Read the model definition and answer for the solid it produces. Units are mm, in the model's axes. Face numbers are marked on the shaded views. Give positions to 0.01 mm unless a question says otherwise; leave off trailing zeros. Loops run counter-clockwise (first coordinate to the right, second up) from the corner with the lowest first, then second, coordinate; pieces in that order, holes last. Notation, with made-up numbers: (66, 46) -> (105, 46) arc R13 cw to (105, 52) -> close; hole circle Ø10 at (-27.75, 63.5). An arc over 180 degrees is marked (long way). Write each question's results on one line, items separated by ' | '. Start each with the question number.
Item 1: Each of these flat-tipped pins is pushed along its axis until it touches: P1, Ø9, axis at x = 21, y = 34.3, coming from the +Z side; P2, Ø2.5, axis at x = 73.5, y = 6, coming from the +Z side. Where does it stop, or does it pass through?
Item 2: Section C-C on z = -6.5 is taken. State how many separate pieces and enclosed holes the cut face has, and give its area (3 significant figures).
Item 3: Section B-B on y = 21.8 is taken. Write down the section's boundary in (x, z), and give its area (3 significant figures).
Item 4: Section A-A on x = 21 is taken. Write down the section's boundary in (y, z).
Item 5: Find the intervals of material crossed by line 1 (Y direction, x = 75, z = -2.1); line 2 (Y direction, x = 36.5, z = -3); line 3 (X direction, y = 9, z = -2), in increasing order.
Item 6: Determine the mould class of the marked faces 1, 2 and 3 for opening direction X: +X half, -X half, draft (parallel to the pull), parting line (faces both ways), or undercut.
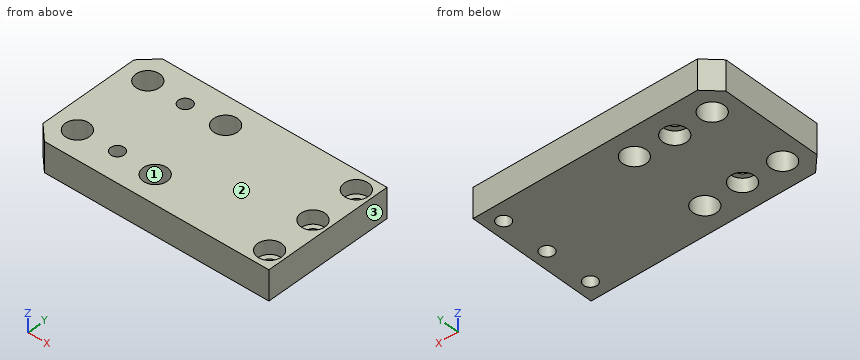
```python
from build123d import *

# Parameters (mm, degrees)
SKETCH_1_W                   = 80
SKETCH_1_H                   = 10
EXTRUDE_1_DEPTH              = 43.6
CHAMFER_1_SIZE               = 5
HOLE_WIZARD_8_0_8_1_D        = 8
HOLE_WIZARD_M4_1_D           = 4.5
HOLE_WIZARD_M4_1_CBORE_D     = 8
HOLE_WIZARD_M4_1_CBORE_DEPTH = 4.6
HOLE_WIZARD_M4_2_D           = 4.5
HOLE_WIZARD_M4_2_CBORE_D     = 8
HOLE_WIZARD_M4_2_CBORE_DEPTH = 4.6


with BuildPart() as part:
    # 草图1 → 凸台-拉伸1 (new body)
    with BuildSketch(Plane(origin=(0, 0, 0), x_dir=(1, 0, 0), z_dir=(0, 1, 0))):
        with Locations((40, 5)):
            Rectangle(SKETCH_1_W, SKETCH_1_H)
    extrude(amount=EXTRUDE_1_DEPTH)

    # 倒角1
    chamfer_1_edges = [part.edges().sort_by_distance(p)[0] for p in [
        (0, 43.6, -5),
        (0, 0, -5),
    ]]
    chamfer(chamfer_1_edges, length=CHAMFER_1_SIZE)

    # Ø8.0 (8) 直径孔1 (through all)
    with Locations(Plane(origin=(0, 0, -10), x_dir=(-1, 0, 0), z_dir=(0, 0, -1))):
        with Locations((-34.042753413, 34.8), (-8.042753413, 34.8), (-8.042753413, 8.8), (-34.042753413, 8.8)):
            Hole(HOLE_WIZARD_8_0_8_1_D / 2)

    # M4 六角圆柱头螺钉的柱形沉头孔1 (through all)
    with Locations(Plane(origin=(0, 0, -10), x_dir=(-1, 0, 0), z_dir=(0, 0, -1))):
        with Locations((-21, 34.3), (-21, 9.3)):
            CounterBoreHole(HOLE_WIZARD_M4_1_D / 2, HOLE_WIZARD_M4_1_CBORE_D / 2, HOLE_WIZARD_M4_1_CBORE_DEPTH)

    # M4 六角圆柱头螺钉的柱形沉头孔2 (through all)
    with Locations(Plane.XY):
        with Locations((75, 37.8), (75, 5.8), (75, 21.8)):
            CounterBoreHole(HOLE_WIZARD_M4_2_D / 2, HOLE_WIZARD_M4_2_CBORE_D / 2, HOLE_WIZARD_M4_2_CBORE_DEPTH)


solid = part.part
```
Findings:
1) P1: z = 0 | P2: z = -4.6
2) separate pieces: 1 | enclosed holes: 9 | area: 3,110 mm2
3) outline: (0, -10) -> (72.75, -10) -> (72.75, -4.6) -> (71, -4.6) -> (71, 0) -> (0, 0) -> close; (77.25, -10) -> (80, -10) -> (80, 0) -> (79, 0) -> (79, -4.6) -> (77.25, -4.6) -> close | area: 739 mm2
4) outline: (0, -10) -> (5.3, -10) -> (5.3, -5.4) -> (7.05, -5.4) -> (7.05, 0) -> (0, 0) -> close; (11.55, -5.4) -> (13.3, -5.4) -> (13.3, -10) -> (30.3, -10) -> (30.3, -5.4) -> (32.05, -5.4) -> (32.05, 0) -> (11.55, 0) -> close; (36.55, -5.4) -> (38.3, -5.4) -> (38.3, -10) -> (43.6, -10) -> (43.6, 0) -> (36.55, 0) -> close
5) line 1: 0 to 1.8, 9.8 to 17.8, 25.8 to 33.8, 41.8 to 43.6 | line 2: 0 to 5.64, 11.96 to 31.64, 37.96 to 43.6 | line 3: 0 to 4.05, 12.04 to 18.77, 23.23 to 30.05, 38.04 to 72.6, 77.4 to 80
6) face 1: undercut | face 2: draft | face 3: +X half
